The figure shows three views and two pictorial views of one solid part (mm, origin at its lowest corner). Answer the questions. A direction names the side the tool comes from. Round coordinates to 2 decimals unless told otherwise and drop trailing zeros. Loops run counter-clockwise (first coordinate to the right, second up) from the corner with the lowest first, then second, coordinate; pieces in that order, holes last. Notation, with made-up numbers: (-23.5, -38.75) - (-19.5, -38.75) arc R5 cw to (-19.5, -33.75) - close; hole circle Ø1 at (71.25, 60.5). An arc over 180 degrees is marked (long way). Use one line per item in the form item = value. Start each with the question number.
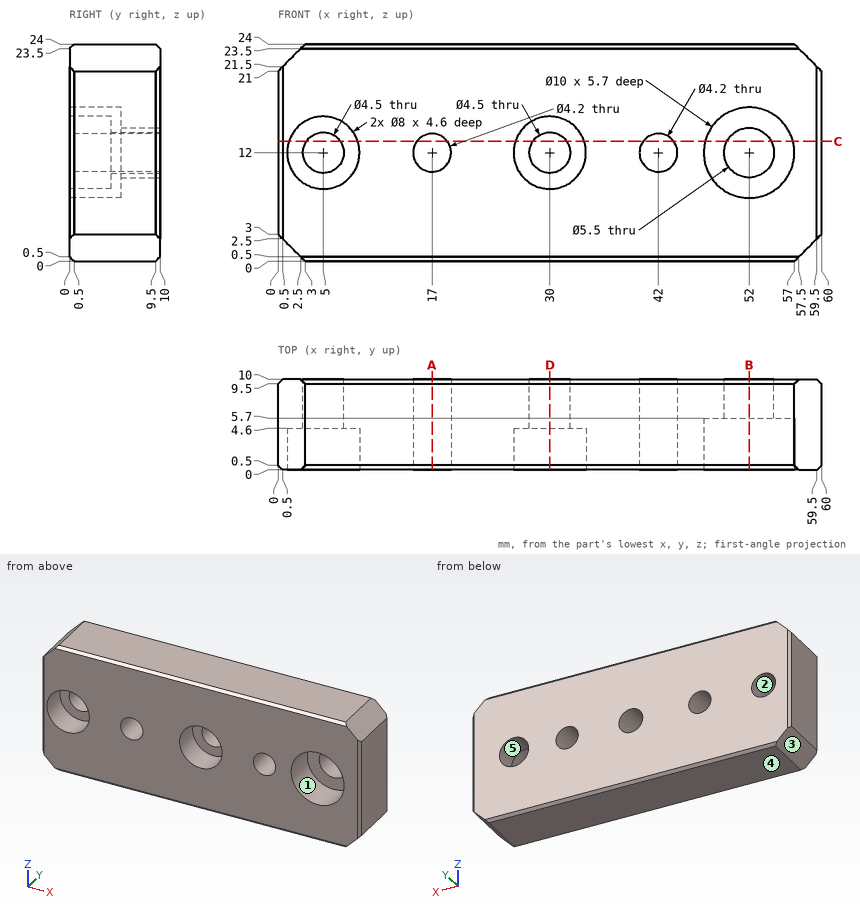
1) A cutting plane is placed at B-B on x = 52. Write down the section's boundary in (y, z), plus the area to 3 significant figures.
2) Determine the mould class of the marked faces 3, 4 and 5 for opening direction X: +X half, -X half, draft (parallel to the pull), parting line (faces both ways), or undercut.
3) A cutting plane is placed at C-C on z = 13.25. Count the separate pieces of the cut face and the enclosed holes in it, plus the area to 3 significant figures.
4) For the marked faces 1 and 2, determine the directions among +Z, -Z, +X, -X, +Y, -Y from which every point of the face is accessible in a straight line to the end or side of a thin tool.
5) Flat-ended cylindrical pins translate along their axes: pin 1 (13 mm diameter, centred on x = 30, z = 12, fed in from +Y); pin 2 (2.5 mm diameter, centred on x = 5, z = 12, fed in from -Y); pin 3 (6.5 mm diameter, centred on x = 52, z = 12, fed in from -Y); pin 4 (6.5 mm diameter, centred on x = 5, z = 12, fed in from -Y). Find the tip coordinate at first contact, or state that the pin passes through.
6) A cutting plane is placed at A-A on x = 17. Write down the section's boundary in (y, z), plus the area to 4 significant figures.
7) A cutting plane is placed at D-D on x = 30. Write down the section's boundary in (y, z).
8) Straight lines are drawn through the part: line 1 (X direction, y = 7.3, z = 12); line 2 (Z direction, x = 17, y = 4.25); line 3 (Z direction, x = 5, y = 3.55). For each, find the intervals that lie inside material, in ascending order. Write a range as from..to.
Checks:
q1.outline = (0, 0.5) - (0.5, 0) - (9.5, 0) - (10, 0.5) - (10, 9.25) - (5.7, 9.25) - (5.7, 7) - (0, 7) - close; (0, 17) - (5.7, 17) - (5.7, 14.75) - (10, 14.75) - (10, 23.5) - (9.5, 24) - (0.5, 24) - (0, 23.5) - close
q1.area = 159 mm²
q2.face_3 = -X half
q2.face_4 = draft
q2.face_5 = undercut
q3.separate_pieces = 6
q3.enclosed_holes = 0
q3.area = 345 mm²
q4.face_1 = -Y
q4.face_2 = +Y, -Y
q5.pin_1 = 10
q5.pin_2 = through
q5.pin_3 = 5.7
q5.pin_4 = 4.6
q6.outline = (0, 0.5) - (0.5, 0) - (9.5, 0) - (10, 0.5) - (10, 9.9) - (0, 9.9) - close; (0, 14.1) - (10, 14.1) - (10, 23.5) - (9.5, 24) - (0.5, 24) - (0, 23.5) - close
q6.area = 197.5 mm²
q7.outline = (0, 0.5) - (0.5, 0) - (9.5, 0) - (10, 0.5) - (10, 9.75) - (4.6, 9.75) - (4.6, 8) - (0, 8) - close; (0, 16) - (4.6, 16) - (4.6, 14.25) - (10, 14.25) - (10, 23.5) - (9.5, 24) - (0.5, 24) - (0, 23.5) - close
q8.line_1 = 0..2.75, 7.25..14.9, 19.1..27.75, 32.25..39.9, 44.1..49.25, 54.75..60
q8.line_2 = 0..9.9, 14.1..24
q8.line_3 = 0..8, 16..24
